from build123d import *

# Parameters (mm, degrees)
SKETCH_1_W                   = 62
SKETCH_1_H                   = 20
EXTRUDE_1_DEPTH              = 8
HOLE_WIZARD_M4_1_D           = 4.5
HOLE_WIZARD_M4_1_CBORE_D     = 8
HOLE_WIZARD_M4_1_CBORE_DEPTH = 4.4
CHAMFER_1_SIZE               = 0.3


with BuildPart() as part:
    # 草图1 → 凸台-拉伸1 (new body)
    with BuildSketch(Plane(origin=(0, 0, 0), x_dir=(1, 0, 0), z_dir=(0, 1, 0))):
        Rectangle(SKETCH_1_W, SKETCH_1_H)
    extrude(amount=EXTRUDE_1_DEPTH)

    # M4 六角凹头螺钉的柱形沉头孔1 (through all)
    with Locations(Plane(origin=(0, 8, 0), x_dir=(1, 0, 0), z_dir=(0, 1, 0))):
        with Locations((-25, -5), (0, -5), (25, -5)):
            CounterBoreHole(HOLE_WIZARD_M4_1_D / 2, HOLE_WIZARD_M4_1_CBORE_D / 2, HOLE_WIZARD_M4_1_CBORE_DEPTH)

    # 倒角1
    chamfer_1_edges = [part.edges().sort_by_distance(p)[0] for p in [
        (-31, 8, 0),
        (0, 8, 10),
        (31, 8, 0),
        (0, 0, 10),
        (-31, 0, 0),
        (0, 0, -10),
        (31, 0, 0),
        (0, 8, -10),
        (31, 4, 10),
        (-31, 4, 10),
        (-31, 4, -10),
        (31, 4, -10),
    ]]
    chamfer(chamfer_1_edges, length=CHAMFER_1_SIZE)


solid = part.part
Design review of the part built by this model. Coordinates are the model's own, in mm. A direction names the side the tool comes from. Round coordinates to 2 decimals unless told otherwise and drop trailing zeros. Write each loop counter-clockwise with the first axis right and the second up, starting at its lowest first coordinate (ties: lowest second). Pieces come first, ordered by that corner, then holes. Notation, with made-up numbers: (-7.75, 46.25) -> (30.25, 46.25) arc R25 ccw to (30.25, 62.25) -> close; hole circle Ø11 at (64, 82.5). An arc over 180 degrees is marked (long way). One line per item, written item: value. Start each with the question number.
Q1. The part is to be moulded in two halves that separate along Z. For faces 3 (the face through (0, 4, 10)), 4 (the face through (31, 4, 0)), 5 (the face through (21.8, 5.8, 7.4)), 6 (the face through (0, 4, -10)), say which applies: pulls with the +Z half, pulls with the -Z half, needs draft (parallel to the pull), parting line crosses it, or undercut.
Q2. To check wall thickness, follow probe 1 along Z at (x, y) = (25, 2.8); probe 2 along Z at (x, y) = (-25, 6.75); probe 3 along X at (y, z) = (4, 3.5). State the ranges of each line that lie inside material, in increasing order.
Q3. Add section D-D (y = 6). Give the boundary of the cut face in (x, z), then the cut area to 3 significant figures.
Q4. Add section A-A (x = 0). Give the boundary of the cut face in (y, z), then the cut area to 3 significant figures.
Q5. Add section B-B (z = 5). State how many separate pieces and enclosed holes the cut face has, then the cut area to 3 significant figures.
Q6. Tool access review of faces 1 (the face through (27, 3.6, 7)), 2 (the face through (22.854, 1.775, 4.324)): name each direction out of +Z, -Z, +X, -X, +Y, -Y from which nothing blocks a thin tool from reaching the whole face with its end or side.
Q7. Insertion check: P1, Ø2.5, axis at x = 25, z = 3.5, coming from the +Y side; P2, Ø2.5, axis at x = 0, z = 5, coming from the -Y side. Each pin has a flat end and moves straight along its axis. Give the tip position at first contact, or say it passes through.
Q8. Add section C-C (y = 2). Give the boundary of the cut face in (x, z).
Response:
1. face 3: pulls with the +Z half
1. face 4: needs draft
1. face 5: undercut
1. face 6: pulls with the -Z half
2. probe 1: z = -10 to 2.75, 7.25 to 10
2. probe 2: z = -10 to 1, 9 to 10
2. probe 3: x = -31 to -28.71, -21.29 to -3.71, 3.71 to 21.29, 28.71 to 31
3. outline: (-31, -9.7) -> (-30.7, -10) -> (30.7, -10) -> (31, -9.7) -> (31, 9.7) -> (30.7, 10) -> (-30.7, 10) -> (-31, 9.7) -> close; hole circle Ø8 at (-25, 5); hole circle Ø8 at (0, 5); hole circle Ø8 at (25, 5)
3. area: 1,090 mm^2
4. outline: (0, -9.7) -> (0.3, -10) -> (7.7, -10) -> (8, -9.7) -> (8, 1) -> (3.6, 1) -> (3.6, 2.75) -> (0, 2.75) -> close; (0, 7.25) -> (3.6, 7.25) -> (3.6, 9) -> (8, 9) -> (8, 9.7) -> (7.7, 10) -> (0.3, 10) -> (0, 9.7) -> close
4. area: 108 mm^2
5. separate pieces: 4
5. enclosed holes: 0
5. area: 342 mm^2
6. face 1: +Y
6. face 2: +Y, -Y
7. P1: stops at y = 3.6
7. P2: passes through
8. outline: (-31, -9.7) -> (-30.7, -10) -> (30.7, -10) -> (31, -9.7) -> (31, 9.7) -> (30.7, 10) -> (-30.7, 10) -> (-31, 9.7) -> close; hole circle Ø4.5 at (-25, 5); hole circle Ø4.5 at (0, 5); hole circle Ø4.5 at (25, 5)
